Design review of the part shown in the three views and the two pictorial views. Dimensions are in mm from the part's minimum x, y and z. A direction names the side the tool comes from. Coordinates: 2 decimals unless noted, no trailing zeros. Order: outer loops, then holes, each group sorted by start corner. A loop starts at its lowest first (then second) coordinate and runs counter-clockwise, first axis right, second up. Notation, with made-up numbers: (2, 39) - (18, 39) arc R14 cw to (18, 64) - close; hole circle Ø6 at (-29.5, 68). An arc over 180 degrees is marked (long way). One line per item, written item: value. Start each with the question number.
(1) To check wall thickness, follow line 1 along Z through (x, y) = (30, 10.5); line 2 along Z through (x, y) = (56.5, 11.75); line 3 along Z through (x, y) = (45, 15.5). State the ranges of each line that lie inside material, in increasing order.
(2) For the marked faces 5 and 6, list the 3-axis set-ups (+Z, -Z, +X, -X, +Y, -Y) from which the entire face can be reached by the end or side of a thin tool; tool diameter is ignored.
(3) Consider section B-B on y = 11.5. Write out the cut boundary in (x, z).
(4) Mouldability with a two-part tool opening along X and no side actions: class the marked faces 1, 2, 3 and 4 as released by +X, released by -X, zero draft, split by the parting line, or undercut.
(5) Clearance check with flat-ended pins moving along their axes: pin 1 (2.5 mm diameter, centred on y = 14.5, z = 8, fed in from -X); pin 2 (5 mm diameter, centred on x = 5.5, y = 21.5, fed in from -Z); pin 3 (5.5 mm diameter, centred on y = 11, z = 1.5, fed in from +X). State where each tip first meets the part, or that it passes through.
(6) Consider section A-A on x = 43.5. Write out the cut boundary in (y, z).
(7) Consider section C-C on x = 52.5. Write out the cut boundary in (y, z).
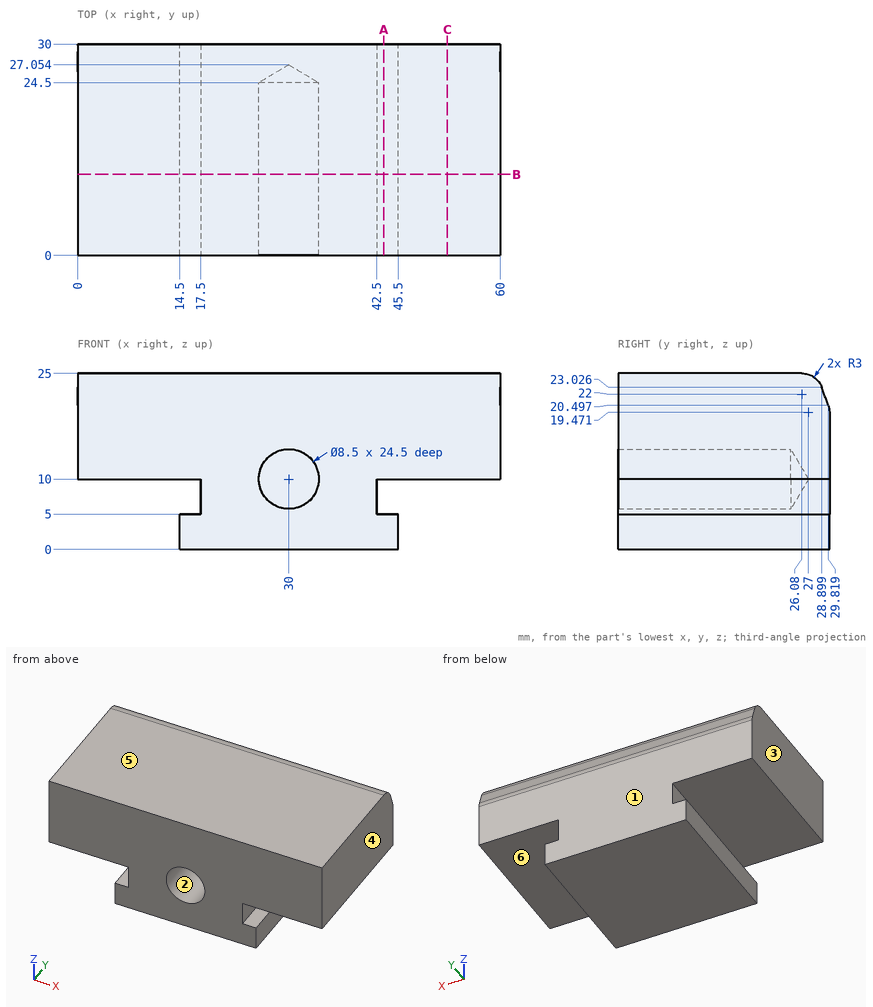
Geometry check:
1. line 1: z = 0 to 5.75, 14.25 to 25
1. line 2: z = 10 to 25
1. line 3: z = 0 to 5, 10 to 25
2. face 5: +Z, +X, -X, +Y, -Y
2. face 6: +X, +Y, -Y
3. outline: (0, 10) - (17.5, 10) - (17.5, 5) - (14.5, 5) - (14.5, 0) - (45.5, 0) - (45.5, 5) - (42.5, 5) - (42.5, 10) - (60, 10) - (60, 25) - (0, 25) - close; hole circle Ø8.5 at (30, 10)
4. face 1: zero draft
4. face 2: undercut
4. face 3: released by -X
4. face 4: released by +X
5. pin 1: stops at x = 17.5
5. pin 2: stops at z = 10
5. pin 3: stops at x = 45.5
6. outline: (0, 0) - (30, 0) - (30, 5) - (0, 5) - close; (0, 10) - (30, 10) - (30, 19.47) arc R3 ccw to (29.82, 20.5) - (28.9, 23.03) arc R3 ccw to (26.08, 25) - (0, 25) - close
7. outline: (0, 10) - (30, 10) - (30, 19.47) arc R3 ccw to (29.82, 20.5) - (28.9, 23.03) arc R3 ccw to (26.08, 25) - (0, 25) - close
